Here's how the part is built. I have some questions about the finished solid (model axes, mm). Face numbers are marked on the shaded views. A direction names the side the tool comes from. Coordinates: 2 decimals unless noted, no trailing zeros. Order: outer loops, then holes, each group sorted by start corner. A loop starts at its lowest first (then second) coordinate and runs counter-clockwise, first axis right, second up. Notation, with made-up numbers: M -13,46.25 L 42,46.25 A7 ccw 42,55.25 Z; hole C -20,76 d3. An arc over 180 degrees is marked long. Answer as CSV lines item,"result". Start each with the question number.
```python
from build123d import *

# Parameters (mm, degrees)
BOSS_EXTRUDE1_DEPTH = 10
BOSS_EXTRUDE2_START = -20
BOSS_EXTRUDE2_DEPTH = 20
BOSS_EXTRUDE3_DEPTH = 10
SKETCH6_W           = 47.967212756
SKETCH6_H           = 31.917124467
CUT_EXTRUDE1_DEPTH  = 1
CUT_EXTRUDE2_DEPTH  = 10


with BuildPart() as part:
    # Sketch2 → Boss-Extrude1 (new body)
    with BuildSketch(Plane.XY):
        with BuildLine():
            Line((567.746058529, 114.079925051), (622.940708708, 67.071408889))
            ThreePointArc((622.940708708, 67.071408889), (633.205576943, 40.118894124), (616.005456238, 16.96805354))
            ThreePointArc((616.005456238, 16.96805354), (587.978717163, -9.525484834), (581.845382902, -47.601565115))
            Line((581.845382902, -47.601565115), (588.918006227, -89.508939159))
            Line((588.918006227, -89.508939159), (603.708844125, -87.012719162))
            Line((603.708844125, -87.012719162), (596.6362208, -45.105345118))
            ThreePointArc((596.6362208, -45.105345118), (601.237559856, -16.539976295), (622.263729898, 3.335958661))
            ThreePointArc((622.263729898, 3.335958661), (648.063910956, 38.062219537), (632.666608603, 78.490991685))
            Line((632.666608603, 78.490991685), (577.471958425, 125.499507846))
            Line((577.471958425, 125.499507846), (567.746058529, 114.079925051))
        make_face()
    extrude(amount=-BOSS_EXTRUDE1_DEPTH)

    # Sketch3 → Boss-Extrude2 (add)
    with BuildSketch(Plane.XY.offset(5).offset(BOSS_EXTRUDE2_START)):
        with BuildLine():
            Line((608.971952758, -88.152757549), (601.566500099, -44.273271785))
            ThreePointArc((601.566500099, -44.273271785), (605.657174086, -18.878140116), (624.349821118, -1.208072965))
            ThreePointArc((624.349821118, -1.208072965), (653.01668896, 37.376661342), (635.908575235, 82.297519283))
            Line((635.908575235, 82.297519283), (567.391078462, 140.652918656))
            ThreePointArc((567.391078462, 140.652918656), (549.769842886, 139.241516239), (551.181245303, 121.620280664))
            Line((551.181245303, 121.620280664), (619.698742076, 63.264881291))
            ThreePointArc((619.698742076, 63.264881291), (628.252798938, 40.80445232), (613.919365017, 21.512085166))
            ThreePointArc((613.919365017, 21.512085166), (583.559102933, -7.187321014), (576.915103602, -48.433638447))
            Line((576.915103602, -48.433638447), (584.320556261, -92.313124211))
            Line((584.320556261, -92.313124211), (608.971952758, -88.152757549))
        make_face()
        with BuildLine():
            Line((577.471958425, 125.499507846), (567.746058529, 114.079925051))
            Line((567.746058529, 114.079925051), (622.940708708, 67.071408889))
            ThreePointArc((622.940708708, 67.071408889), (633.205576943, 40.118894124), (616.005456238, 16.96805354))
            ThreePointArc((616.005456238, 16.96805354), (587.978717163, -9.525484834), (581.845382902, -47.601565115))
            Line((581.845382902, -47.601565115), (588.918006227, -89.508939159))
            Line((588.918006227, -89.508939159), (603.708844125, -87.012719162))
            Line((603.708844125, -87.012719162), (596.6362208, -45.105345118))
            ThreePointArc((596.6362208, -45.105345118), (601.237559856, -16.539976295), (622.263729898, 3.335958661))
            ThreePointArc((622.263729898, 3.335958661), (648.063910956, 38.062219537), (632.666608603, 78.490991685))
            Line((632.666608603, 78.490991685), (577.471958425, 125.499507846))
        make_face(mode=Mode.SUBTRACT)
        with BuildLine():
            ThreePointArc((558.45408855, 136.066878959), (554.355882583, 130.304526327), (560.118235215, 126.20632036))
            ThreePointArc((560.118235215, 126.20632036), (564.216441182, 131.968672992), (558.45408855, 136.066878959))
        make_face(mode=Mode.SUBTRACT)
    extrude(amount=BOSS_EXTRUDE2_DEPTH)

    # Sketch4 → Boss-Extrude3 (add)
    with BuildSketch(Plane.XY.offset(-5)):
        with BuildLine():
            Line((608.696660412, -86.521569404), (584.013862627, -90.495874195))
            Line((584.013862627, -90.495874195), (586.899983592, -107.596990039))
            ThreePointArc((586.899983592, -107.596990039), (601.305865171, -117.842504957), (611.551380088, -103.436623377))
            Line((611.551380088, -103.436623377), (608.696660412, -86.521569404))
        make_face()
        with BuildLine():
            ThreePointArc((598.393608507, -100.586527409), (594.295402541, -106.348880041), (600.057755172, -110.447086008))
            ThreePointArc((600.057755172, -110.447086008), (604.155961139, -104.684733376), (598.393608507, -100.586527409))
        make_face(mode=Mode.SUBTRACT)
    extrude(amount=-BOSS_EXTRUDE3_DEPTH)

    # Sketch6 → Cut-Extrude1 (cut)
    with BuildSketch(Plane(origin=(0, 0, -15), x_dir=(-1, 0, 0), z_dir=(0, 0, -1))):
        with Locations((-595.88807181, -104.755141446)):
            Rectangle(SKETCH6_W, SKETCH6_H)
    extrude(amount=-CUT_EXTRUDE1_DEPTH, mode=Mode.SUBTRACT)

    # Sketch7 → Cut-Extrude2 (cut)
    with BuildSketch(Plane.XY.offset(5)):
        Polygon((608.971952758, -88.152757549), (584.051383166, -90.718194429), (584.320556261, -92.313124211), align=None)
    extrude(amount=-CUT_EXTRUDE2_DEPTH, mode=Mode.SUBTRACT)


solid = part.part
```
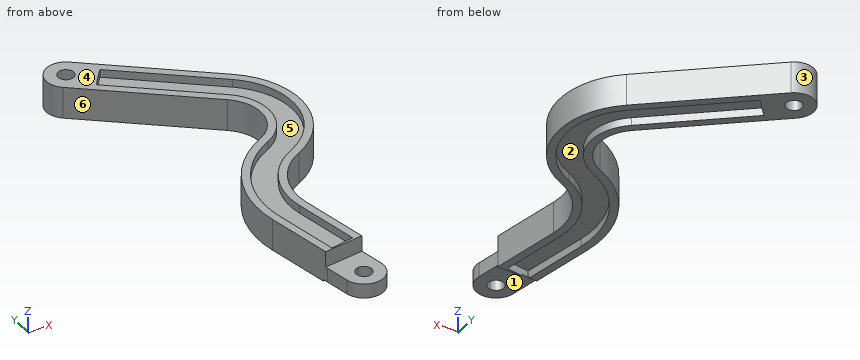
1) Which directions (+Z, -Z, +X, -X, +Y, -Y) give clear straight access to the entire face, cutting with the end or side of a thin tool? Please do the marked faces 1, 2 and 3.
2) If we mould it in two halves opening along X, with no side actions, what happens to the marked faces 4, 5 and 6? For each: released by +X, released by -X, zero draft, split by the parting line, or undercut.
3) Suppose I cut it at C-C on y = -52.5. Please give me the cut outline in (x, z), plus the area to 3 significant figures.
4) Suppose I cut it at A-A on z = 2.5. Please give me the cut outline in (x, y).
5) Suppose I cut it at B-B on y = 34. Please give me the cut outline in (x, z), plus the area to 3 significant figures.
6) I need wall thicknesses on line 1 (Z direction, x = 633.5, y = 46.5); line 2 (X direction, y = 5, z = -12.5); line 3 (Y direction, x = 611.5, z = 1.5). Which ranges of each line are inside material? Lowest first, please. Write a range as [from, to].
7) Will these pins go through, and if not, where does the flat tip stop? pin 1 Ø10 at (x, z) = (606, -0.5) entering from -Y; pin 2 Ø12 at (x, z) = (575.5, -2) entering from +Y; pin 3 Ø14 at (x, y) = (594, -110) entering from +Z.
Output:
1,face 1,"-Z, +X, -X, -Y"
1,face 2,"-Z"
1,face 3,"+Z, -Z"
2,face 4,"zero draft"
2,face 5,"undercut"
2,face 6,"released by -X"
3,outline,"M 577.6,-15 L 582.67,-15 L 582.67,-10 L 597.88,-10 L 597.88,-15 L 602.95,-15 L 602.95,5 L 597.88,5 L 597.88,0 L 582.67,0 L 582.67,5 L 577.6,5 Z"
3,area,"355 mm²"
4,outline,"M 551.18,121.62 L 619.7,63.26 A25 cw 613.92,21.51 A65.05 ccw 576.92,-48.43 L 584.05,-90.72 L 608.97,-88.15 L 601.57,-44.27 A40.05 cw 624.35,-1.21 A50 ccw 635.91,82.3 L 567.39,140.65 A12.5 ccw Z; hole C 559.29,131.14 d10; hole M 567.75,114.08 L 622.94,67.07 A30 cw 616.01,16.97 A60.05 ccw 581.85,-47.6 L 588.92,-89.51 L 603.71,-87.01 L 596.64,-45.11 A45.05 cw 622.26,3.34 A45 ccw 632.67,78.49 L 577.47,125.5 Z"
5,outline,"M 626.3,-15 L 631.69,-15 L 631.69,-10 L 647.31,-10 L 647.31,-15 L 652.43,-15 L 652.43,5 L 647.31,5 L 647.31,0 L 631.69,0 L 631.69,5 L 626.3,5 Z"
5,area,"366 mm²"
6,line 1,"[-10, 0]"
6,line 2,"[591.9, 598.74], [625.53, 634.49]"
6,line 3,"[-10.58, -3.61], [14.67, 20.34], [70.25, 76.82], [96.52, 103.09]"
7,pin 1,"y = -117.14"
7,pin 2,"y = 138.86"
7,pin 3,"z = -5"
